```python
from build123d import *

# Parameters (mm, degrees)
SKETCH1_W                  = 35
SKETCH1_H                  = 30
BOSS_EXTRUDE1_DEPTH        = 2
SKETCH2_W                  = 10
SKETCH2_H                  = 15
CUT_EXTRUDE1_DEPTH         = 24.393375131
F_3_0_3_DIAMETER_HOLE2_D   = 3
F_3_0_3_DIAMETER_HOLE1_D   = 3
F_4_5_4_5_DIAMETER_HOLE1_D = 4.5
CHAMFER1_SIZE              = 1
CUT_EXTRUDE2_DEPTH         = 24.393375131


with BuildPart() as part:
    # Sketch1 → Boss-Extrude1 (new, symmetric)
    with BuildSketch(Plane.XY):
        Rectangle(SKETCH1_W, SKETCH1_H)
    extrude(amount=BOSS_EXTRUDE1_DEPTH, both=True)

    # Sketch2 → Cut-Extrude1 (cut, through all)
    with BuildSketch(Plane.XY.offset(2)):
        with Locations((12.5, -7.5)):
            Rectangle(SKETCH2_W, SKETCH2_H)
    extrude(amount=-CUT_EXTRUDE1_DEPTH, mode=Mode.SUBTRACT)

    # Ø3.0 (3) Diameter Hole2 (through all)
    with Locations(Plane.XY.offset(2)):
        with Locations((7.5, 0)):
            Hole(F_3_0_3_DIAMETER_HOLE2_D / 2)

    # Ø3.0 (3) Diameter Hole1 (through all)
    with Locations(Plane.XY.offset(2)):
        with Locations((-12.5, 9), (-12.5, -9)):
            Hole(F_3_0_3_DIAMETER_HOLE1_D / 2)

    # Ø4.5 (4.5) Diameter Hole1 (through all)
    with Locations(Plane.XY.offset(2)):
        with Locations((-2.5, 9), (-2.5, -9)):
            Hole(F_4_5_4_5_DIAMETER_HOLE1_D / 2)

    # Chamfer1
    chamfer1_edges = [part.edges().sort_by_distance(p)[0] for p in [
        (17.5, 0, 0),
        (7.5, -15, 0),
        (-17.5, -15, 0),
        (-17.5, 15, 0),
        (17.5, 15, 0),
    ]]
    chamfer(chamfer1_edges, length=CHAMFER1_SIZE)

    # Sketch9 → Cut-Extrude2 (cut, through all)
    with BuildSketch(Plane.XY.offset(2)):
        with BuildLine():
            Line((-11, 9.25), (-11, 8.75))
            ThreePointArc((-11, 8.75), (-12.5, 7.25), (-14, 8.75))
            Line((-14, 8.75), (-14, 9.25))
            ThreePointArc((-14, 9.25), (-12.5, 10.75), (-11, 9.25))
        make_face()
    extrude(amount=-CUT_EXTRUDE2_DEPTH, mode=Mode.SUBTRACT)


solid = part.part
```
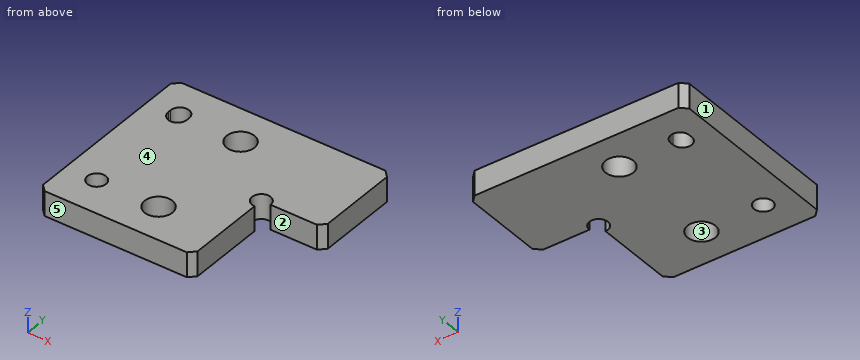
Geometry check sheet. Reference: the model listing, model coordinates, mm. Face numbers are marked on the shaded views. A direction names the side the tool comes from. Coordinates: 2 decimals unless noted, no trailing zeros. Order: outer loops, then holes, each group sorted by start corner. A loop starts at its lowest first (then second) coordinate and runs counter-clockwise, first axis right, second up. Notation, with made-up numbers: (-39, 0) - (7, 0) arc R14 cw to (7, 26) - close; hole circle Ø7 at (3, 67.25). An arc over 180 degrees is marked (long way). Answer as a JSON object with one key per item and string values. Group by question number.
Item 1: Depth check by flat-ended pin: pin 1 Ø1.5 at (y, z) = (-5, 1.5) entering from +X; pin 2 Ø2.5 at (x, y) = (-12.5, -9) entering from -Z; pin 3 Ø2 at (x, z) = (11, -1) entering from -Y. Enter the tip coordinate at first touch or a pass-through.
Item 2: Tool access check on the marked faces 1 and 2. Record the directions out of +Z, -Z, +X, -X, +Y, -Y that give a thin tool (end or side, any length) a straight path to the whole face; none if there is none.
Item 3: Sectioned sample at C-C, the plane z = -0.3. Record the cut outline in (x, y), and give its area (3 significant figures).
Item 4: Draft check along Y on the marked faces 3, 4 and 5. Enter one of: +Y half, -Y half, draft (parallel to the pull), parting line (faces both ways), or undercut.
Item 5: Sectioned sample at D-D, the plane x = 13. Record the cut outline in (y, z), and give its area (3 significant figures).
Item 6: Sectioned sample at B-B, the plane x = -12.5. Record the cut outline in (y, z), and give its area (3 significant figures).
Item 7: Scan lines: probe 1 along Y at (x, z) = (-2.5, 0.9); probe 2 along Y at (x, z) = (-12.5, 0.3); probe 3 along X at (y, z) = (10, -1.1). Record each from-to range of solid material in increasing order.
Item 8: Sectioned sample at A-A, the plane y = -9. Record the cut outline in (x, z).
Resolved:
{
 "1": {"pin 1": "x = 7.5", "pin 2": "through", "pin 3": "y = 0"},
 "2": {"face 1": "+Z, -Z, -X, +Y, -Y", "face 2": "+Z, -Z, +X, -Y"},
 "3": {"outline": "(-17.5, -14) - (-16.5, -15) - (6.5, -15) - (7.5, -14) - (7.5, -1.5) arc R1.5 cw (long way) to (9, 0) - (16.5, 0) - (17.5, 1) - (17.5, 14) - (16.5, 15) - (-16.5, 15) - (-17.5, 14) - close; hole circle Ø3 at (-12.5, -9); hole (-14, 8.75) arc R1.5 ccw to (-11, 8.75) - (-11, 9.25) arc R1.5 ccw to (-14, 9.25) - close; hole circle Ø4.5 at (-2.5, -9); hole circle Ø4.5 at (-2.5, 9)", "area": "845 mm^2"},
 "4": {"face 3": "undercut", "face 4": "draft", "face 5": "-Y half"},
 "5": {"outline": "(0, -2) - (15, -2) - (15, 2) - (0, 2) - close", "area": "60.0 mm^2"},
 "6": {"outline": "(-15, -2) - (-10.5, -2) - (-10.5, 2) - (-15, 2) - close; (-7.5, -2) - (7.25, -2) - (7.25, 2) - (-7.5, 2) - close; (10.75, -2) - (15, -2) - (15, 2) - (10.75, 2) - close", "area": "94.0 mm^2"},
 "7": {"probe 1": "-15 to -11.25, -6.75 to 6.75, 11.25 to 15", "probe 2": "-15 to -10.5, -7.5 to 7.25, 10.75 to 15", "probe 3": "-17.5 to -13.8, -11.2 to -4.52, -0.48 to 17.5"},
 "8": {"outline": "(-17.5, -2) - (-14, -2) - (-14, 2) - (-17.5, 2) - close; (-11, -2) - (-4.75, -2) - (-4.75, 2) - (-11, 2) - close; (-0.25, -2) - (7.5, -2) - (7.5, 2) - (-0.25, 2) - close"}
}
